Could you check a few things on this model? Use its own coordinates, in mm. A direction names the side the tool comes from. Round coordinates to 2 decimals unless told otherwise and drop trailing zeros. Loops run counter-clockwise (first coordinate to the right, second up) from the corner with the lowest first, then second, coordinate; pieces in that order, holes last.
from build123d import *

# Parameters (mm, degrees)
SKETCH1_R           = 50
SKETCH1_R_2         = 3.5
SKETCH1_R_3         = 18
BOSS_EXTRUDE1_DEPTH = 8
SKETCH2_R           = 27.5
SKETCH2_R_2         = 18
BOSS_EXTRUDE2_DEPTH = 10
SKETCH3_R           = 25
SKETCH3_R_2         = 18
BOSS_EXTRUDE3_DEPTH = 16


with BuildPart() as part:
    # Sketch1 → Boss-Extrude1 (new body)
    with BuildSketch(Plane.XY):
        Circle(SKETCH1_R)
        with Locations((0, 42.5)):
            Circle(SKETCH1_R_2, mode=Mode.SUBTRACT)
        with Locations((-36.806079661, -21.25)):
            Circle(SKETCH1_R_2, mode=Mode.SUBTRACT)
        with Locations((36.806079661, -21.25)):
            Circle(SKETCH1_R_2, mode=Mode.SUBTRACT)
        Circle(SKETCH1_R_3, mode=Mode.SUBTRACT)
    extrude(amount=BOSS_EXTRUDE1_DEPTH)

    # Sketch2 → Boss-Extrude2 (add)
    with BuildSketch(Plane.XY.offset(8)):
        Circle(SKETCH2_R)
        Circle(SKETCH2_R_2, mode=Mode.SUBTRACT)
    extrude(amount=BOSS_EXTRUDE2_DEPTH)

    # Sketch3 → Boss-Extrude3 (add)
    with BuildSketch(Plane.XY.offset(18)):
        Circle(SKETCH3_R)
        Circle(SKETCH3_R_2, mode=Mode.SUBTRACT)
    extrude(amount=BOSS_EXTRUDE3_DEPTH)


solid = part.part
Item 1: If we section it at C-C, the plane z = 4: Please give me the cut outline in (x, y), then the cut area to 3 significant figures.
Results list:
outline: circle Ø100 at (0, 0); hole circle Ø7 at (-36.81, -21.25); hole circle Ø36 at (0, 0); hole circle Ø7 at (0, 42.5); hole circle Ø7 at (36.81, -21.25)
area: 6,720 mm2
Item 2: Will these pins go through, and if not, where does the flat tip stop? pin 1 (3 mm diameter, centred on x = -6, y = -32, fed in from +Z); pin 2 (10 mm diameter, centred on x = -1, z = 10.5, fed in from -Y); pin 3 (16.5 mm diameter, centred on x = -4.5, y = 2, fed in from +Z); pin 4 (12 mm diameter, centred on x = -12.5, z = 27, fed in from +Y).
Results list:
pin 1: stops at z = 8
pin 2: stops at y = -50
pin 3: passes through
pin 4: stops at y = 24.14
Item 3: If we section it at D-D, the plane y = -21.25: Please give me the cut outline in (x, z).
Results list:
outline: (-45.26, 0) - (-40.31, 0) - (-40.31, 8) - (-45.26, 8) - close; (-33.31, 0) - (33.31, 0) - (33.31, 8) - (17.46, 8) - (17.46, 18) - (13.17, 18) - (13.17, 34) - (-13.17, 34) - (-13.17, 18) - (-17.46, 18) - (-17.46, 8) - (-33.31, 8) - close; (40.31, 0) - (45.26, 0) - (45.26, 8) - (40.31, 8) - close
Item 4: If I drill on line 1 along Y through (x, z) = (0, 5.25); line 2 along X through (y, z) = (-0.5, 12); line 3 along Y through (x, z) = (0, 9), over which ranges is the centre line in solid material (lowest first)?
Results list:
line 1: y = -50 to -18, 18 to 39, 46 to 50
line 2: x = -27.5 to -17.99, 17.99 to 27.5
line 3: y = -27.5 to -18, 18 to 27.5
Item 5: If we section it at A-A, the plane x = 0: Please give me the cut outline in (y, z), then the cut area to 3 significant figures.
Results list:
outline: (-50, 0) - (-18, 0) - (-18, 34) - (-25, 34) - (-25, 18) - (-27.5, 18) - (-27.5, 8) - (-50, 8) - close; (18, 0) - (39, 0) - (39, 8) - (27.5, 8) - (27.5, 18) - (25, 18) - (25, 34) - (18, 34) - close; (46, 0) - (50, 0) - (50, 8) - (46, 8) - close
area: 870 mm2
Item 6: If we section it at B-B, the plane y = 0: Please give me the cut outline in (x, z), then the cut area to 3 significant figures.
Results list:
outline: (-50, 0) - (-18, 0) - (-18, 34) - (-25, 34) - (-25, 18) - (-27.5, 18) - (-27.5, 8) - (-50, 8) - close; (18, 0) - (50, 0) - (50, 8) - (27.5, 8) - (27.5, 18) - (25, 18) - (25, 34) - (18, 34) - close
area: 926 mm2
Item 7: We'd pull the mould along X, two halves only. Please class faces 1 (the flat face through (22, -22, 8)), 2 (the cylindrical face through (23.846, 7.509, 25.888)), 3 (the cylindrical face through (-2.343, 17.847, 16.762)): released by +X, released by -X, zero draft, split by the parting line, or undercut.
Results list:
face 1: zero draft
face 2: split by the parting line
face 3: undercut
Item 8: For faces 4 (the cylindrical face through (-5.961, -26.846, 12.93)), 5 (the flat face through (11, -16, 34)), which set-ups out of +Z, -Z, +X, -X, +Y, -Y let a thin tool reach every point of the face, with its end or its side?
Results list:
face 4: +Z
face 5: +Z, +X, -X, +Y, -Y
